Design review of the part built by this model. Coordinates are the model's own, in mm. A direction names the side the tool comes from. Give positions to 0.01 mm unless a question says otherwise; leave off trailing zeros. Loops run counter-clockwise (first coordinate to the right, second up) from the corner with the lowest first, then second, coordinate; pieces in that order, holes last. Notation, with made-up numbers: (-20.75, 58.25) - (34.25, 58.25) arc R20 ccw to (34.25, 70.25) - close; hole circle Ø3 at (-15, -14). An arc over 180 degrees is marked (long way). Put each result on its own line as item: value. Start each with the question number.
```python
from build123d import *

# Parameters (mm, degrees)
SKETCH1_R              = 95
SKETCH1_R_2            = 67.5
BOSS_EXTRUDE1_DEPTH    = 10
SKETCH2_R              = 90
SKETCH2_R_2            = 67.5
BOSS_EXTRUDE2_DEPTH    = 15
M12_TAPPED_HOLE2_D     = 10.2
M12_TAPPED_HOLE2_DEPTH = 10
M12_TAPPED_HOLE2_TIP   = 3.064389157


with BuildPart() as part:
    # Sketch1 → Boss-Extrude1 (new body)
    with BuildSketch(Plane.XY):
        Circle(SKETCH1_R)
        Circle(SKETCH1_R_2, mode=Mode.SUBTRACT)
    extrude(amount=BOSS_EXTRUDE1_DEPTH)

    # Sketch2 → Boss-Extrude2 (add)
    with BuildSketch(Plane.XY.offset(10)):
        Circle(SKETCH2_R)
        Circle(SKETCH2_R_2, mode=Mode.SUBTRACT)
    extrude(amount=BOSS_EXTRUDE2_DEPTH)

    # M12 Tapped Hole2
    with Locations(Plane(origin=(0, 80.5, 0), x_dir=(-1, 0, 0), z_dir=(0, 0, -1))):
        with Locations((0, 0), (-69.715045005, -40.25), (-69.715045005, -120.75), (0, -161), (69.715045005, -120.75), (69.715045005, -40.25)):
            Hole(M12_TAPPED_HOLE2_D / 2, depth=M12_TAPPED_HOLE2_DEPTH)
            with Locations((0, 0, -(M12_TAPPED_HOLE2_DEPTH + M12_TAPPED_HOLE2_TIP / 2))):  # 118° drill point
                Cone(0, M12_TAPPED_HOLE2_D / 2, M12_TAPPED_HOLE2_TIP, mode=Mode.SUBTRACT)


solid = part.part
```
Item 1: Consider section C-C (x = -33.5). State the section outline as (y, z) points, plus the area to 3 significant figures.
Item 2: Mouldability with a two-part tool opening along X and no side actions: class faces 4 (the conical face through (0.192, 79.635, 12.532)), 5 (the cylindrical face through (41.53, -79.845, 17.395)), 6 (the flat face through (13, 67, 25)) as pulls with the +X half, pulls with the -X half, needs draft (parallel to the pull), parting line crosses it, or undercut.
Item 3: For L1, parallel to X at y = 40.25, z = 6.75; L2, parallel to X at y = 39, z = 9; L3, parallel to Y at x = 32, z = 22, list the stretches that pass through material, from the lowest coordinate up. Write a range as from..to.
Item 4: Consider section B-B (y = 0). State the section outline as (x, z) points, plus the area to 4 significant figures.
Item 5: Consider section A-A (z = 5.25). State the section outline as (x, y) points, plus the area to 3 significant figures.
Item 6: Machinability: for faces 1 (the cylindrical face through (-20.59, -92.74, 4.93)), 2 (the cylindrical face through (-0.664, -75.443, 5.07)), 3 (the flat face through (-57, -70, 10)), which of the approach directions +Z, -Z, +X, -X, +Y, -Y give a long, thin tool a straight path to every point of the face, cutting with its end or side? Answer none if there is none.
Item 7: For P1, Ø10, axis at y = 62.5, z = 4, coming from the +X side; P2, Ø8, axis at x = 74.5, z = 16, coming from the -Y side; P3, Ø3, axis at x = -71, z = 18, coming from the +Y side, all flat-tipped, find the tip position at first contact; note any pin that passes through.
Item 8: Consider section D-D (z = 15.25). State the section outline as (x, y) points, plus the area to 3 significant figures.
Geometry says:
1. outline: (-88.9, 0) - (-58.6, 0) - (-58.6, 25) - (-83.53, 25) - (-83.53, 10) - (-88.9, 10) - close; (58.6, 0) - (88.9, 0) - (88.9, 10) - (83.53, 10) - (83.53, 25) - (58.6, 25) - close
1. area: 1,350 mm2
2. face 4: undercut
2. face 5: parting line crosses it
2. face 6: needs draft
3. L1: x = -86.05..-74.82, -64.62..-54.19, 54.19..64.62, 74.82..86.05
3. L2: x = -86.63..-74.66, -64.77..-55.09, 55.09..64.77, 74.66..86.63
3. L3: y = -84.12..-59.43, 59.43..84.12
4. outline: (-95, 0) - (-67.5, 0) - (-67.5, 25) - (-90, 25) - (-90, 10) - (-95, 10) - close; (67.5, 0) - (95, 0) - (95, 10) - (90, 10) - (90, 25) - (67.5, 25) - close
4. area: 1,225 mm2
5. outline: circle Ø190 at (0, 0); hole circle Ø10.2 at (-69.72, -40.25); hole circle Ø10.2 at (-69.72, 40.25); hole circle Ø135 at (0, 0); hole circle Ø10.2 at (0, -80.5); hole circle Ø10.2 at (0, 80.5); hole circle Ø10.2 at (69.72, -40.25); hole circle Ø10.2 at (69.72, 40.25)
5. area: 13,500 mm2
6. face 1: +Z, -Z
6. face 2: -Z
6. face 3: +Z
7. P1: stops at x = 75.62
7. P2: stops at y = -55.94
7. P3: stops at y = 57.18
8. outline: circle Ø180 at (0, 0); hole circle Ø135 at (0, 0)
8. area: 11,100 mm2
